Check sheet for the modelled part. Datum: model origin and axes. Units: mm. Face numbers are marked on the shaded views. A direction names the side the tool comes from. Round coordinates to 2 decimals unless told otherwise and drop trailing zeros. Order: outer loops, then holes, each group sorted by start corner. A loop starts at its lowest first (then second) coordinate and runs counter-clockwise, first axis right, second up. Notation, with made-up numbers: (73.5, 51) -> (128.5, 51) arc R18 ccw to (128.5, 62) -> close; hole circle Ø2 at (33.25, 53.25). An arc over 180 degrees is marked (long way). Answer in a Markdown table with one row per item. Add a question column.
1. Sectioned sample at D-D, the plane y = -18. Record the boundary of the cut face in (x, z), then the cut area to 3 significant figures.
2. Sectioned sample at B-B, the plane z = 0. Record the boundary of the cut face in (x, y).
3. Sectioned sample at C-C, the plane x = -20. Record the boundary of the cut face in (y, z).
4. Material ranges on L1, parallel to X at y = 5, z = 25; L2, parallel to Z at x = 20, y = -20; L3, parallel to Z at x = -20, y = 34, recorded low to high. Write a range as from..to.
5. Draft check along Y on the marked faces 1, 2 and 3. Enter one of: +Y half, -Y half, draft (parallel to the pull), parting line (faces both ways), or undercut.
6. Sectioned sample at A-A, the plane y = 8. Record the boundary of the cut face in (x, z), then the cut area to 3 significant figures.
7. Access from +Z, -Z, +X, -X, +Y, -Y to the whole of each face (thin tool, end or side, straight path). Record for the marked faces 4 and 5.
8. Depth check by flat-ended pin: P1, Ø21, axis at y = 6.5, z = 6.5, coming from the +X side; P2, Ø3.5, axis at x = 22, z = 22.5, coming from the +Y side. Enter the tip coordinate at first touch or a pass-through.
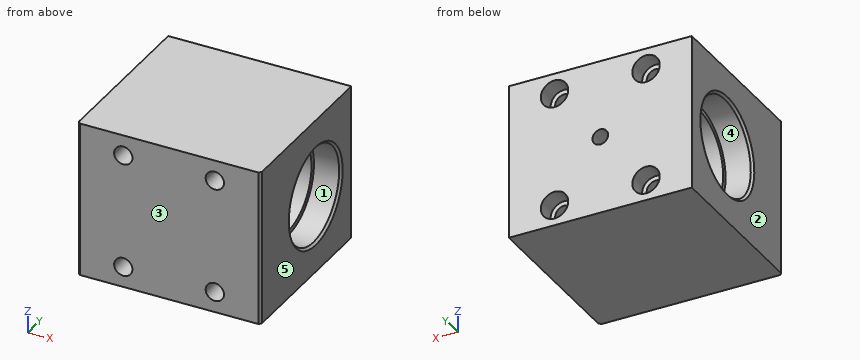
```python
from build123d import *

# Parameters (mm, degrees)
SKETCH1_W                                            = 40
SKETCH1_H                                            = 68
BOSS_EXTRUDE1_DEPTH                                  = 37
M8_TAPPED_HOLE1_D                                    = 6.8
M8_TAPPED_HOLE1_DEPTH                                = 30
M8_TAPPED_HOLE1_TIP                                  = 2.042926105
SKETCH11_R                                           = 21
CUT_EXTRUDE4_DEPTH                                   = 12
SKETCH12_R                                           = 19
CUT_EXTRUDE5_DEPTH                                   = 85.551759296
CHAMFER1_SIZE                                        = 1
CHAMFER3_SIZE                                        = 1
HOLE_SIZE_PER_SOCKET_HEAD_CAP_SCREW_TYPE_D           = 8
HOLE_SIZE_PER_SOCKET_HEAD_CAP_SCREW_TYPE_CBORE_D     = 12
HOLE_SIZE_PER_SOCKET_HEAD_CAP_SCREW_TYPE_CBORE_DEPTH = 8
MIRROR5_COPY_1_D                                     = 8
MIRROR5_COPY_1_CBORE_D                               = 12
MIRROR5_COPY_1_CBORE_DEPTH                           = 8


with BuildPart() as part:
    # Sketch1 → Boss-Extrude1 (new, symmetric)
    with BuildSketch(Plane(origin=(0, 0, 0), x_dir=(1, 0, 0), z_dir=(0, 1, 0))):
        with Locations((20, 0)):
            Rectangle(SKETCH1_W, SKETCH1_H)
    extrude(amount=BOSS_EXTRUDE1_DEPTH, both=True)

    # Mirror2: part across plane


with BuildPart() as part_1:
    add(part.part)
    add(part.part.mirror(Plane(origin=(0, 37, 0), x_dir=(0, 0, 1), z_dir=(-1, 0, 0))))

    # M8 Tapped Hole1
    with Locations(Plane(origin=(0, 37, 0), x_dir=(1, 0, 0), z_dir=(0, 1, 0))):
        with Locations((0, 0)):
            Hole(M8_TAPPED_HOLE1_D / 2, depth=M8_TAPPED_HOLE1_DEPTH)
            with Locations((0, 0, -(M8_TAPPED_HOLE1_DEPTH + M8_TAPPED_HOLE1_TIP / 2))):  # 118° drill point
                Cone(0, M8_TAPPED_HOLE1_D / 2, M8_TAPPED_HOLE1_TIP, mode=Mode.SUBTRACT)

    # Sketch11 → Cut-Extrude4 (cut)
    with BuildSketch(Plane(origin=(40, 0, 0), x_dir=(0, 0, -1), z_dir=(1, 0, 0))):
        with Locations((0, 8)):
            Circle(SKETCH11_R)
    cut_extrude4 = extrude(amount=-CUT_EXTRUDE4_DEPTH, mode=Mode.SUBTRACT)

    # Mirror3: Cut-Extrude4 across plane
    add(cut_extrude4.mirror(Plane(origin=(0, 0, 0), x_dir=(0, 0, 1), z_dir=(1, 0, 0))), mode=Mode.SUBTRACT)

    # Sketch12 → Cut-Extrude5 (cut, through all)
    with BuildSketch(Plane(origin=(28, 0, 0), x_dir=(0, 0, -1), z_dir=(1, 0, 0))):
        with Locations((0, 8)):
            Circle(SKETCH12_R)
    extrude(amount=-CUT_EXTRUDE5_DEPTH, mode=Mode.SUBTRACT)

    # Chamfer1
    chamfer1_edges = [part_1.edges().sort_by_distance(p)[0] for p in [
        (40, 8, 21),
        (-40, 8, 21),
    ]]
    chamfer(chamfer1_edges, length=CHAMFER1_SIZE)

    # Chamfer3
    chamfer3_edges = [part_1.edges().sort_by_distance(p)[0] for p in [
        (-40, -37, 0),
        (40, -37, 0),
    ]]
    chamfer(chamfer3_edges, length=CHAMFER3_SIZE)

    # Hole size per socket head cap screw type1 (through all)
    with Locations(Plane(origin=(0, 37, 0), x_dir=(1, 0, 0), z_dir=(0, 1, 0))):
        with Locations((-20, -25)):
            hole_size_per_socket_head_cap_screw_type = CounterBoreHole(HOLE_SIZE_PER_SOCKET_HEAD_CAP_SCREW_TYPE_D / 2, HOLE_SIZE_PER_SOCKET_HEAD_CAP_SCREW_TYPE_CBORE_D / 2, HOLE_SIZE_PER_SOCKET_HEAD_CAP_SCREW_TYPE_CBORE_DEPTH)

    # Mirror4: Hole size per socket head cap screw type1 across plane
    add(hole_size_per_socket_head_cap_screw_type.mirror(Plane.XY), mode=Mode.SUBTRACT)

    # Mirror5: Hole size per socket head cap screw type1 across plane
    add(hole_size_per_socket_head_cap_screw_type.mirror(Plane(origin=(0, 0, 0), x_dir=(0, 0, 1), z_dir=(1, 0, 0))), mode=Mode.SUBTRACT)

    # Mirror5 copy 1 (through all)
    with Locations(Plane(origin=(0, 37, 0), x_dir=(-1, 0, 0), z_dir=(0, 1, 0))):
        with Locations((-20, -25)):
            CounterBoreHole(MIRROR5_COPY_1_D / 2, MIRROR5_COPY_1_CBORE_D / 2, MIRROR5_COPY_1_CBORE_DEPTH)


solid = part_1.part
```
Answer key:
| question | item | result |
|---|---|---|
| 1 | outline | (-40, -34) -> (40, -34) -> (40, 34) -> (-40, 34) -> close; hole circle Ø8 at (-20, -25); hole circle Ø8 at (-20, 25); hole circle Ø8 at (20, -25); hole circle Ø8 at (20, 25) |
| 1 | area | 5,240 mm² |
| 2 | outline | (-40, -36) -> (-39, -37) -> (39, -37) -> (40, -36) -> (40, -14) -> (39, -13) -> (28, -13) -> (28, -11) -> (-28, -11) -> (-28, -13) -> (-39, -13) -> (-40, -14) -> close; (-40, 30) -> (-39, 29) -> (-28, 29) -> (-28, 27) -> (-3.4, 27) -> (-3.4, 37) -> (-40, 37) -> close; (3.4, 27) -> (28, 27) -> (28, 29) -> (39, 29) -> (40, 30) -> (40, 37) -> (3.4, 37) -> close |
| 3 | outline | (-37, -34) -> (37, -34) -> (37, -31) -> (29, -31) -> (29, -29) -> (-37, -29) -> close; (-37, -21) -> (29, -21) -> (29, -19) -> (37, -19) -> (37, 19) -> (29, 19) -> (29, 21) -> (-37, 21) -> close; (-37, 29) -> (29, 29) -> (29, 31) -> (37, 31) -> (37, 34) -> (-37, 34) -> close; hole circle Ø38 at (8, 0) |
| 4 | L1 | x = -40..-24, -16..16, 24..40 |
| 4 | L2 | z = -34..-29, -21..21, 29..34 |
| 4 | L3 | z = -34..-31, -19..19, 31..34 |
| 5 | face 1 | undercut |
| 5 | face 2 | draft |
| 5 | face 3 | -Y half |
| 6 | outline | (-40, -34) -> (40, -34) -> (40, -22) -> (39, -21) -> (28, -21) -> (28, -19) -> (-28, -19) -> (-28, -21) -> (-39, -21) -> (-40, -22) -> close; (-40, 22) -> (-39, 21) -> (-28, 21) -> (-28, 19) -> (28, 19) -> (28, 21) -> (39, 21) -> (40, 22) -> (40, 34) -> (-40, 34) -> close; hole circle Ø8 at (-20, -25); hole circle Ø8 at (-20, 25); hole circle Ø8 at (20, -25); hole circle Ø8 at (20, 25) |
| 6 | area | 2,100 mm² |
| 7 | face 4 | -X |
| 7 | face 5 | +Z, -Z, +X, +Y, -Y |
| 8 | P1 | passes through |
| 8 | P2 | stops at y = 29 |
